CAD build for the part. Positions are in the model's coordinates, mm. A direction names the side the tool comes from. Give positions to 0.01 mm unless a question says otherwise; leave off trailing zeros. Write each loop counter-clockwise with the first axis right and the second up, starting at its lowest first coordinate (ties: lowest second). Pieces come first, ordered by that corner, then holes. Notation, with made-up numbers: M -36,15 L -17,15 A19 cw -17,41 Z; hole C 6.5,-25.75 d5. An arc over 180 degrees is marked long. One line per question, with ' | ' between items. Start each with the question number.
1. Pull direction X, two halves, no side cores. Call faces 6 (the face through (39.08, 41.28, 58.04)), 7 (the face through (25, 45, 34)), 8 (the face through (10.92, 41.28, 57.96)), 9 (the face through (39.004, 35.341, 42.748)): released by +X, released by -X, zero draft, split by the parting line, or undercut.
2. Which spindle directions (+Z, -Z, +X, -X, +Y, -Y) get a long thin tool onto all of the face, cutting with end or side? Do faces 1 (the face through (50, 22, 34)), 2 (the face through (0, 22, 34)), 3 (the face through (44.879, 42.115, 56.784)), 4 (the face through (3.69, 7.5, 5.12)), 5 (the face through (20, 4, 61)). Say none if no direction does.
3. Flat gauge pins, fed straight in: pin 1 (1.5 mm diameter, centred on y = 37, z = 10.5, fed in from -X); pin 2 (21 mm diameter, centred on x = 16, y = 23.5, fed in from +Z); pin 3 (2 mm diameter, centred on y = 41, z = 58, fed in from -X); pin 4 (2 mm diameter, centred on x = 27, y = 5, fed in from +Z) (1 decimal). Where does each tip first touch, or does it go through?
4. Wall check: L1, parallel to Z at x = 6.5, y = 41; L2, parallel to Y at x = 25.5, z = 22; L3, parallel to X at y = 5.5, z = 31. Give the ranges that are in metal, low to high.
5. Cut at C-C, the plane z = 6. Write the cut outline in (x, y).
6. Cut at B-B, the plane y = 22.5. Write the cut outline in (x, z), then the cut area to 3 significant figures.
7. Cut at D-D, the plane x = 18.5. Write the cut outline in (y, z).
8. Cut at A-A, the plane x = 8.5. Write the cut outline in (y, z).
```python
from build123d import *

# Parameters (mm, degrees)
SKETCH_1_W                  = 50
SKETCH_1_H                  = 45
EXTRUDE_1_DEPTH             = 68
SKETCH_2_R                  = 19
CUT_EXTRUDE_1_DEPTH         = 79
SKETCH_3_R                  = 21
CUT_EXTRUDE_2_DEPTH         = 7
CUT_EXTRUDE_START           = -25
SKETCH_4_R                  = 21
CUT_EXTRUDE_3_DEPTH         = 25
HOLE_WIZARD_M4_1_D          = 3.3
HOLE_WIZARD_M4_1_DEPTH      = 10.1
HOLE_WIZARD_M4_1_TIP        = 0.991420021
HOLE_WIZARD_M4_2_D          = 3.3
HOLE_WIZARD_M4_2_DEPTH      = 10.1
HOLE_WIZARD_M4_2_TIP        = 0.991420021
HOLE_WIZARD_6_5_6_5_1_D     = 6.5
HOLE_WIZARD_6_5_6_5_1_DEPTH = 20
HOLE_WIZARD_6_5_6_5_1_TIP   = 1.952797012
HOLE_WIZARD_M4_4_D          = 3.3
HOLE_WIZARD_M4_4_DEPTH      = 10.1
HOLE_WIZARD_M4_4_TIP        = 0.991420021


with BuildPart() as part:
    # 草图1 → 凸台-拉伸1 (new body)
    with BuildSketch(Plane.XY):
        with Locations((25, 22.5)):
            Rectangle(SKETCH_1_W, SKETCH_1_H)
    extrude(amount=EXTRUDE_1_DEPTH)

    # 草图2 → 切除-拉伸1 (cut)
    with BuildSketch(Plane(origin=(0, 0, 0), x_dir=(-1, 0, 0), z_dir=(0, 0, -1))):
        with Locations((-25, 22.5)):
            Circle(SKETCH_2_R)
    extrude(amount=-CUT_EXTRUDE_1_DEPTH, mode=Mode.SUBTRACT)

    # 草图3 → 切除-拉伸2 (cut)
    with BuildSketch(Plane.XY.offset(68)):
        with Locations((25, 22.5)):
            Circle(SKETCH_3_R)
    extrude(amount=-CUT_EXTRUDE_2_DEPTH, mode=Mode.SUBTRACT)

    # 草图4 → 切除-拉伸3 (cut)
    with BuildSketch(Plane(origin=(0, 0, 0), x_dir=(-1, 0, 0), z_dir=(0, 0, -1)).offset(CUT_EXTRUDE_START)):
        with Locations(Location((-25, 22.5, 0), (0, 0, 180))):
            Circle(SKETCH_4_R)
    extrude(amount=CUT_EXTRUDE_3_DEPTH, mode=Mode.SUBTRACT)

    # M4 螺纹孔1
    with Locations(Plane(origin=(50, 0, 0), x_dir=(0, 0, -1), z_dir=(1, 0, 0))):
        with Locations((-58, 41), (-46, 41)):
            Hole(HOLE_WIZARD_M4_1_D / 2, depth=HOLE_WIZARD_M4_1_DEPTH)
            with Locations((0, 0, -(HOLE_WIZARD_M4_1_DEPTH + HOLE_WIZARD_M4_1_TIP / 2))):  # 118° drill point
                Cone(0, HOLE_WIZARD_M4_1_D / 2, HOLE_WIZARD_M4_1_TIP, mode=Mode.SUBTRACT)

    # M4 螺纹孔2
    with Locations(Plane.ZY):
        with Locations((46, 41), (58, 41)):
            Hole(HOLE_WIZARD_M4_2_D / 2, depth=HOLE_WIZARD_M4_2_DEPTH)
            with Locations((0, 0, -(HOLE_WIZARD_M4_2_DEPTH + HOLE_WIZARD_M4_2_TIP / 2))):  # 118° drill point
                Cone(0, HOLE_WIZARD_M4_2_D / 2, HOLE_WIZARD_M4_2_TIP, mode=Mode.SUBTRACT)

    # Ø6.5 (6.5) 直径孔1
    with Locations(Plane(origin=(0, 0, 0), x_dir=(-1, 0, 0), z_dir=(0, -1, 0))):
        with Locations((-25, -38)):
            Hole(HOLE_WIZARD_6_5_6_5_1_D / 2, depth=HOLE_WIZARD_6_5_6_5_1_DEPTH)
            with Locations((0, 0, -(HOLE_WIZARD_6_5_6_5_1_DEPTH + HOLE_WIZARD_6_5_6_5_1_TIP / 2))):  # 118° drill point
                Cone(0, HOLE_WIZARD_6_5_6_5_1_D / 2, HOLE_WIZARD_6_5_6_5_1_TIP, mode=Mode.SUBTRACT)

    # M4 螺纹孔4
    with Locations(Plane(origin=(0, 0, 0), x_dir=(-1, 0, 0), z_dir=(0, 0, -1))):
        with Locations((-5, 36.5), (-45, 36.5), (-45, 8.5), (-5, 8.5)):
            Hole(HOLE_WIZARD_M4_4_D / 2, depth=HOLE_WIZARD_M4_4_DEPTH)
            with Locations((0, 0, -(HOLE_WIZARD_M4_4_DEPTH + HOLE_WIZARD_M4_4_TIP / 2))):  # 118° drill point
                Cone(0, HOLE_WIZARD_M4_4_D / 2, HOLE_WIZARD_M4_4_TIP, mode=Mode.SUBTRACT)


solid = part.part
```
Here are the results:
1) face 6: released by +X | face 7: zero draft | face 8: released by -X | face 9: undercut
2) face 1: +Z, -Z, +X, +Y, -Y | face 2: +Z, -Z, -X, +Y, -Y | face 3: +X | face 4: -Z | face 5: +Z
3) pin 1: x = 0 | pin 2: z = 61 | pin 3: x = 10.49 | pin 4: through
4) L1: 0 to 44.35, 47.65 to 56.35, 59.65 to 68 | L2: 0 to 1.51, 43.49 to 45 | L3: 0 to 16.51, 33.49 to 50
5) outline: M 0,0 L 50,0 L 50,45 L 0,45 Z; hole C 5,8.5 d3.3; hole C 5,36.5 d3.3; hole C 25,22.5 d42; hole C 45,8.5 d3.3; hole C 45,36.5 d3.3
6) outline: M 0,0 L 4,0 L 4,25 L 6,25 L 6,61 L 4,61 L 4,68 L 0,68 Z; M 44,25 L 46,25 L 46,0 L 50,0 L 50,68 L 46,68 L 46,61 L 44,61 Z | area: 688 mm^2
7) outline: M 0,0 L 2.53,0 L 2.53,25 L 4.65,25 L 4.65,61 L 2.53,61 L 2.53,68 L 0,68 Z; M 40.35,25 L 42.47,25 L 42.47,0 L 45,0 L 45,68 L 42.47,68 L 42.47,61 L 40.35,61 Z
8) outline: M 0,0 L 9.51,0 L 9.51,25 L 13.08,25 L 13.08,61 L 9.51,61 L 9.51,68 L 0,68 Z; M 31.92,25 L 35.49,25 L 35.49,0 L 45,0 L 45,68 L 35.49,68 L 35.49,61 L 31.92,61 Z; hole C 41,46 d3.3; hole C 41,58 d3.3
